from build123d import *

# Parameters (mm, degrees)
GB_T707_1988_18A_XXXXXXXXXXXXXXX528V9_2_DEPTH = 500
CUT_EXTRUDE_1_DEPTH                           = 536.746208573
HOLE_WIZARD_16_0_16_1_REACH                   = 537.746
HOLE_WIZARD_16_0_16_1_BORE_R                  = 8


with BuildPart() as part:
    # Sketch11 → 热轧普通槽钢(gb t707-1988) 18A-XXXXXXXXXXXXXXX528V9(2) (new body)
    with BuildSketch(Plane(origin=(0, 0, 0), x_dir=(-1, 0, 0), z_dir=(0, 1, 0))):
        with BuildLine():
            Line((68, 180), (0, 180))
            Line((0, 180), (0, 0))
            Line((0, 0), (68, 0))
            Line((68, 0), (68, 2.698815299))
            ThreePointArc((68, 2.698815299), (66.642625801, 6.221593233), (63.272394525, 7.922760548))
            Line((63.272394525, 7.922760548), (16.45521095, 12.604478905))
            ThreePointArc((16.45521095, 12.604478905), (9.714748398, 16.006813534), (7, 23.052369402))
            Line((7, 23.052369402), (7, 156.947630598))
            ThreePointArc((7, 156.947630598), (9.714748398, 163.993186466), (16.45521095, 167.395521095))
            Line((16.45521095, 167.395521095), (63.272394525, 172.077239452))
            ThreePointArc((63.272394525, 172.077239452), (66.642625801, 173.778406767), (68, 177.301184701))
            Line((68, 177.301184701), (68, 180))
        make_face()
    extrude(amount=GB_T707_1988_18A_XXXXXXXXXXXXXXX528V9_2_DEPTH)

    # 草图8 → 切除-拉伸1 (cut, through all)
    with BuildSketch(Plane(origin=(0, 0, 180), x_dir=(0, 0, 1), z_dir=(-1, 0, 0))):
        Polygon((0, 500), (-180, 350), (-180, 500), align=None)
        Polygon((-180, 0), (0, 0), (-180, 150), align=None)
    extrude(amount=CUT_EXTRUDE_1_DEPTH, mode=Mode.SUBTRACT)

    # Ø16.0 (16) 直径孔1 bore → Ø16.0 (16) 直径孔1 (cut, up to next)
    with BuildSketch(Plane(origin=(0, 0, 0), x_dir=(-1, 0, 0), z_dir=(0, 0, -1)), mode=Mode.PRIVATE) as hole_wizard_16_0_16_1_sk1:
        with Locations((34, 318)):
            Circle(HOLE_WIZARD_16_0_16_1_BORE_R)
    hole_wizard_16_0_16_1_tool1 = extrude(hole_wizard_16_0_16_1_sk1.sketch, amount=-HOLE_WIZARD_16_0_16_1_REACH, mode=Mode.PRIVATE) & part.part
    # Ø16.0 (16) 直径孔1 bore → Ø16.0 (16) 直径孔1 (cut, up to next)
    with BuildSketch(Plane(origin=(0, 0, 0), x_dir=(-1, 0, 0), z_dir=(0, 0, -1)), mode=Mode.PRIVATE) as hole_wizard_16_0_16_1_sk2:
        with Locations((34, 182)):
            Circle(HOLE_WIZARD_16_0_16_1_BORE_R)
    hole_wizard_16_0_16_1_tool2 = extrude(hole_wizard_16_0_16_1_sk2.sketch, amount=-HOLE_WIZARD_16_0_16_1_REACH, mode=Mode.PRIVATE) & part.part
    add(hole_wizard_16_0_16_1_tool1.solids().sort_by_distance((-34, 318, 0))[0], mode=Mode.SUBTRACT)
    add(hole_wizard_16_0_16_1_tool2.solids().sort_by_distance((-34, 182, 0))[0], mode=Mode.SUBTRACT)


solid = part.part
CAD build for the part. Positions are in the model's coordinates, mm. A direction names the side the tool comes from. Round coordinates to 2 decimals unless told otherwise and drop trailing zeros. Loops run counter-clockwise (first coordinate to the right, second up) from the corner with the lowest first, then second, coordinate; pieces in that order, holes last.
(1) Drop flat-ended pins along their axis: pin 1 (13 mm diameter, centred on x = -34, y = 318, fed in from -Z); pin 2 (14.5 mm diameter, centred on x = -34, y = 182, fed in from -Z) (3 decimals); pin 3 (1 mm diameter, centred on x = -38, y = 367, fed in from -Z). Give the stop position or say it passes through.
(2) Cut at B-B (x = -35). Give the cut face in (y, z), plus the area to 3 significant figures.
(3) Cut at A-A (y = 182). Give the cut face in (x, z), plus the area to 3 significant figures.
(4) Cut at D-D (z = 93). Give the cut face in (x, y), plus the area to 4 significant figures.
(5) Wall check: line 1 along X through (y, z) = (318, 3); line 2 along Y through (x, z) = (-34, 6); line 3 along Y through (x, z) = (-34, 3.25). Give the ranges that are in metal, low to high.
(6) Two-plate mould, pull along Z, no slides. Class faces 4 (the cylindrical face through (-9.788, 248.331, 15.927)), 5 (the flat face through (-34, 249, 0)), 6 (the flat face through (-34, 246, 180)): +Z half, -Z half, draft (parallel to the pull), parting line (faces both ways), or undercut.
(7) Cut at C-C (y = 69.5). Give the cut face in (x, z), plus the area to 3 significant figures.
(8) Which spindle directions (+Z, -Z, +X, -X, +Y, -Y) get a long thin tool onto all of the face, cutting with end or side? Do faces 1 (the flat face through (0, 246, 111)), 2 (the cylindrical face through (-26, 318, 6)), 3 (the flat face through (-39.5, 246.6, 169.7)). Say none if no direction does.
Findings below:
1. pin 1: stops at z = 168.5
1. pin 2: stops at z = 168.425
1. pin 3: stops at z = 169.5
2. outline: (0, 180) - (8.96, 169.25) - (491.04, 169.25) - (500, 180) - close; (141.04, 10.75) - (150, 0) - (174.06, 0) - (174.06, 10.75) - close; (189.94, 0) - (310.06, 0) - (310.06, 10.75) - (189.94, 10.75) - close; (325.94, 0) - (350, 0) - (358.96, 10.75) - (325.94, 10.75) - close
2. area: 7,180 mm2
3. outline: (-68, 0) - (-42, 0) - (-42, 10.05) - (-63.27, 7.92) arc R5.25 ccw to (-68, 2.7) - close; (-68, 177.3) arc R5.25 ccw to (-63.27, 172.08) - (-16.46, 167.4) arc R10.5 cw to (-7, 156.95) - (-7, 23.05) arc R10.5 cw to (-16.46, 12.6) - (-26, 11.65) - (-26, 0) - (0, 0) - (0, 180) - (-68, 180) - close
3. area: 2,400 mm2
4. outline: (-7, 72.5) - (0, 72.5) - (0, 427.5) - (-7, 427.5) - close
4. area: 2,485 mm2
5. line 1: x = -67.99 to -42, -26 to 0
5. line 2: y = 145 to 174, 190 to 310, 326 to 355
5. line 3: y = 147.29 to 174, 190 to 310, 326 to 352.71
6. face 4: undercut
6. face 5: -Z half
6. face 6: +Z half
7. outline: (-68, 177.3) arc R5.25 ccw to (-63.27, 172.08) - (-16.46, 167.4) arc R10.5 cw to (-7, 156.95) - (-7, 96.6) - (0, 96.6) - (0, 180) - (-68, 180) - close
7. area: 1,240 mm2
8. face 1: +Z, -Z, +X, +Y, -Y
8. face 2: -Z
8. face 3: -X, +Y, -Y
